Input: part model. Units: mm. Frame: model coordinates. Coordinates: 2 decimals unless noted, no trailing zeros. Order: outer loops, then holes, each group sorted by start corner. A loop starts at its lowest first (then second) coordinate and runs counter-clockwise, first axis right, second up. Notation, with made-up numbers: M 26.25,81 L 64.25,81 A33 ccw 64.25,111 Z; hole C 87,-36 d1. An arc over 180 degrees is marked long. Answer in a Markdown table with one row per item.
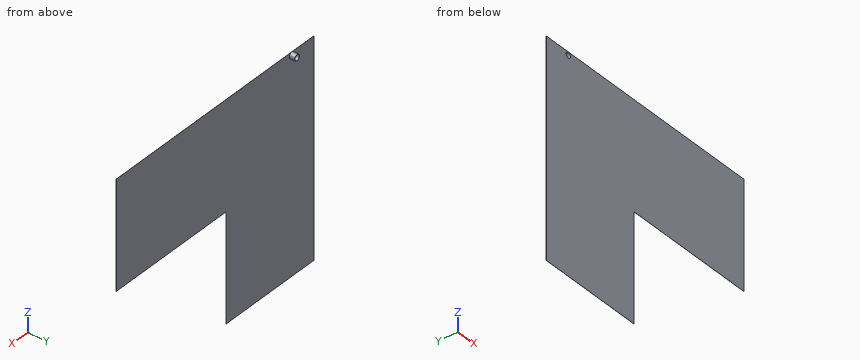
from build123d import *

# Parameters (mm, degrees)
BOSS_EXTRUDE1_DEPTH = 1
SKETCH2_R           = 20
CUT_EXTRUDE1_DEPTH  = 1205.159873107
BOSS_EXTRUDE2_START = 39
SKETCH3_R           = 23.5
SKETCH3_R_2         = 20
BOSS_EXTRUDE2_DEPTH = 39


with BuildPart() as part:
    # Sketch1 → Boss-Extrude1 (new body)
    with BuildSketch(Plane(origin=(0, 0, 0), x_dir=(1, 0, 0), z_dir=(0, 1, 0))):
        Polygon((-900, -800), (900, -800), (900, 0), (0, 0), (-100, 0), (-100, 800), (-900, 800), align=None)
    extrude(amount=BOSS_EXTRUDE1_DEPTH)

    # Sketch2 → Cut-Extrude1 (cut, through all)
    with BuildSketch(Plane(origin=(0, 1, 0), x_dir=(1, 0, 0), z_dir=(0, 1, 0))):
        with Locations(Location((-700, -776.5, 0), (0, 0, 270))):
            Circle(SKETCH2_R)
    extrude(amount=-CUT_EXTRUDE1_DEPTH, mode=Mode.SUBTRACT)

    # Sketch3 → Boss-Extrude2 (add)
    with BuildSketch(Plane(origin=(0, 1, 0), x_dir=(1, 0, 0), z_dir=(0, 1, 0)).offset(BOSS_EXTRUDE2_START)):
        with Locations(Location((-700, -776.5, 0), (0, 0, 270))):
            Circle(SKETCH3_R)
        with Locations(Location((-700, -776.5, 0), (0, 0, 270))):
            Circle(SKETCH3_R_2, mode=Mode.SUBTRACT)
    extrude(amount=-BOSS_EXTRUDE2_DEPTH)


solid = part.part
1) Cut plane B-B, the plane y = 9.5. Output: boundary loops of the cut face in (x, z), and give its area (3 significant figures).
Resolved:
| item | result |
|---|---|
| outline | C -700,776.5 d47; hole C -700,776.5 d40 |
| area | 478 mm2 |
2) Material intervals for probe 1 along X at (y, z) = (13.5, 776.5); probe 2 along Y at (x, z) = (386, 76.5), sorted ascending.
Resolved:
| item | result |
|---|---|
| probe 1 | x = -723.5 to -720, -680 to -676.5 |
| probe 2 | y = 0 to 1 |
3) Cut plane D-D, the plane z = -420.5. Output: boundary loops of the cut face in (x, y), and give its area (3 significant figures).
Resolved:
| item | result |
|---|---|
| outline | M -900,0 L -100,0 L -100,1 L -900,1 Z |
| area | 800 mm2 |
4) Cut plane A-A, the plane z = 776.5. Output: boundary loops of the cut face in (x, y), and give its area (3 significant figures).
Resolved:
| item | result |
|---|---|
| outline | M -900,0 L -720,0 L -720,40 L -723.5,40 L -723.5,1 L -900,1 Z; M -680,0 L 900,0 L 900,1 L -676.5,1 L -676.5,40 L -680,40 Z |
| area | 2,030 mm2 |
5) Contact query for flat-ended pins moving along their axis: pin 1 (5 mm diameter, centred on x = -217.5, z = -197, fed in from +Y); pin 2 (0.5 mm diameter, centred on y = 0.5, z = -423, fed in from +X); pin 3 (1.1 mm diameter, centred on x = 547, y = 0.5, fed in from -Z). Output: stop coordinate, or through.
Resolved:
| item | result |
|---|---|
| pin 1 | stops at y = 1 |
| pin 2 | stops at x = -100 |
| pin 3 | stops at z = 0 |
6) Cut plane C-C, the plane x = 371. Output: boundary loops of the cut face in (y, z), and give its area (3 significant figures).
Resolved:
| item | result |
|---|---|
| outline | M 0,0 L 1,0 L 1,800 L 0,800 Z |
| area | 800 mm2 |
